For this review, use the dimensioned drawing (mm, ordinates from the lowest corner) and the shaded views. A direction names the side the tool comes from. Coordinates: 2 decimals unless noted, no trailing zeros. Loops run counter-clockwise (first coordinate to the right, second up) from the corner with the lowest first, then second, coordinate; pieces in that order, holes last.
1. Take a section at A-A, the plane z = 70. State the section outline as (x, y) points.
2. Clearance check with flat-ended pins moving along their axes: P1, Ø1.5, axis at x = 4.5, z = 90, coming from the -Y side; P2, Ø14, axis at y = 70, z = 20, coming from the +X side; P3, Ø4, axis at x = 10.5, z = 111.5, coming from the +Y side; P4, Ø5, axis at x = 6.5, z = 67.5, coming from the -Y side. State where each tip first meets the part, or that it passes through.
3. To check wall thickness, follow probe 1 along Y at (x, z) = (10, 70); probe 2 along Z at (x, y) = (3.25, 78); probe 3 along X at (y, z) = (124, 29.5). State the ranges of each line that lie inside material, in increasing order.
4. Mouldability with a two-part tool opening along Z and no side actions: class the marked faces 3, 4 and 5 as pulls with the +Z half, pulls with the -Z half, needs draft (parallel to the pull), parting line crosses it, or undercut.
5. Take a section at D-D, the plane z = 120. State the section outline as (x, y) points.
6. Take a section at C-C, the plane x = 10.5. State the section outline as (y, z) points, then the cut area to 3 significant figures.
7. Machinability: for the marked faces 1 and 2, which of the approach directions +Z, -Z, +X, -X, +Y, -Y give a long, thin tool a straight path to every point of the face, cutting with its end or side? Answer none if there is none.
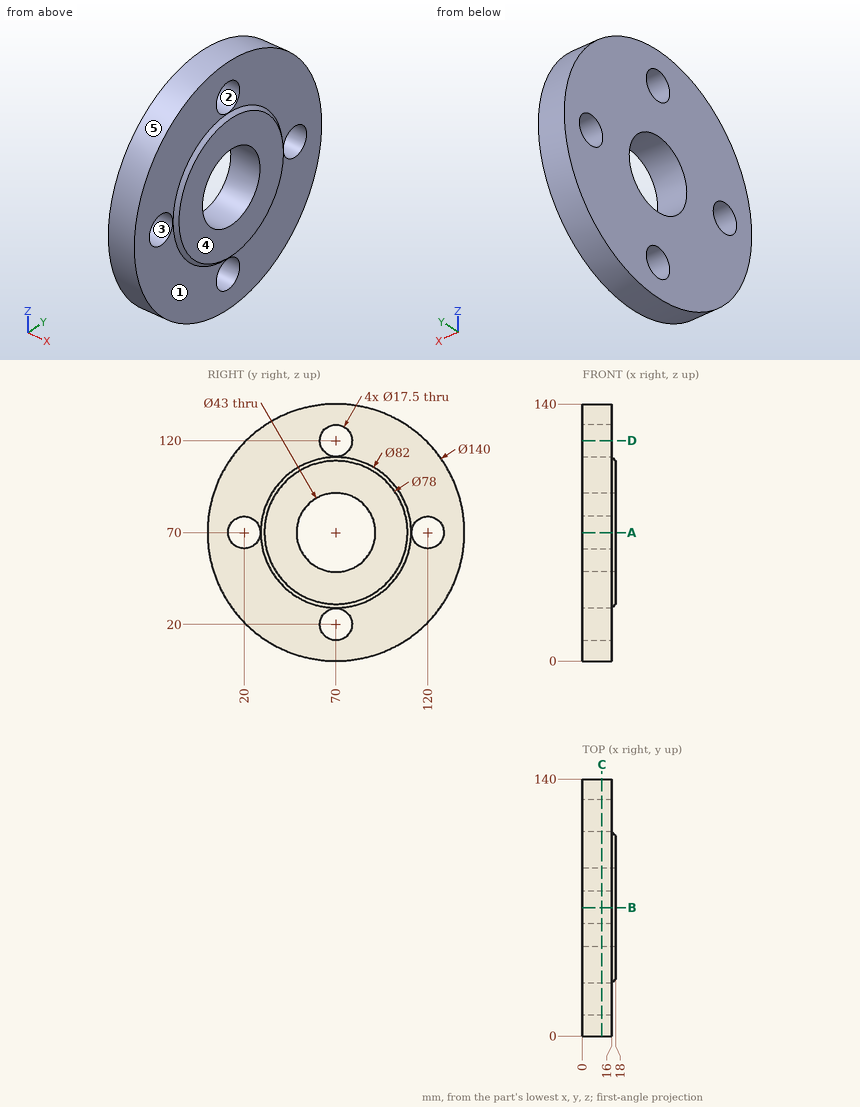
Results list:
1. outline: (0, 0) - (16, 0) - (16, 11.25) - (0, 11.25) - close; (0, 28.75) - (16, 28.75) - (16, 29) - (18, 31) - (18, 48.5) - (0, 48.5) - close; (0, 91.5) - (18, 91.5) - (18, 109) - (16, 111) - (16, 111.25) - (0, 111.25) - close; (0, 128.75) - (16, 128.75) - (16, 140) - (0, 140) - close
2. P1: stops at y = 2.7
2. P2: passes through
2. P3: stops at y = 127.79
2. P4: stops at y = 0
3. probe 1: y = 0 to 11.25, 28.75 to 48.5, 91.5 to 111.25, 128.75 to 140
3. probe 2: z = 0.46 to 16.46, 23.54 to 50.04, 89.96 to 116.46, 123.54 to 139.54
3. probe 3: x = 0 to 16
4. face 3: undercut
4. face 4: needs draft
4. face 5: parting line crosses it
5. outline: (0, 21.01) - (16, 21.01) - (16, 61.25) - (0, 61.25) - close; (0, 78.75) - (16, 78.75) - (16, 118.99) - (0, 118.99) - close
6. outline: circle Ø140 at (70, 70); hole circle Ø17.5 at (20, 70); hole circle Ø43 at (70, 70); hole circle Ø17.5 at (70, 20); hole circle Ø17.5 at (70, 120); hole circle Ø17.5 at (120, 70)
6. area: 13,000 mm2
7. face 1: +X
7. face 2: +X, -X
